CAD build for the part. Positions are in the model's coordinates, mm. Round coordinates to 2 decimals unless told otherwise and drop trailing zeros. Order: outer loops, then holes, each group sorted by start corner. A loop starts at its lowest first (then second) coordinate and runs counter-clockwise, first axis right, second up. Notation, with made-up numbers: M 20.5,57.25 L 39.5,57.25 A23 ccw 39.5,95.25 Z; hole C 37.5,37 d1. An arc over 180 degrees is marked long. Answer as a JSON object with one key per item and string values.
```python
from build123d import *

# Parameters (mm, degrees)
SKETCH1_W                  = 150
SKETCH1_H                  = 260
BOSS_EXTRUDE1_DEPTH        = 10
F_14_0_14_DIAMETER_HOLE1_D = 14


with BuildPart() as part:
    # Sketch1 → Boss-Extrude1 (new body)
    with BuildSketch(Plane.XY):
        Rectangle(SKETCH1_W, SKETCH1_H)
    extrude(amount=BOSS_EXTRUDE1_DEPTH)

    # Ø14.0 (14) Diameter Hole1 (through all)
    with Locations(Plane.XY.offset(10)):
        with Locations((-55, 100), (-55, 0), (-55, -100), (55, -100), (55, 0), (55, 100)):
            Hole(F_14_0_14_DIAMETER_HOLE1_D / 2)


solid = part.part
```
Item 1: Saw through at B-B on z = 7. List the corners of the cut face in (x, y).
Worked answers:
{"outline": "M -75,-130 L 75,-130 L 75,130 L -75,130 Z; hole C -55,-100 d14; hole C -55,0 d14; hole C -55,100 d14; hole C 55,-100 d14; hole C 55,0 d14; hole C 55,100 d14"}
Item 2: Wall check: line 1 along Y through (x, z) = (55, 6); line 2 along Y through (x, z) = (-60.5, 8.5); line 3 along X through (y, z) = (105.5, 6.25). Give the ranges that are in metal, low to high. Write a range as [from, to].
Worked answers:
{"line 1": "y = [-130, -107], [-93, -7], [7, 93], [107, 130]", "line 2": "y = [-130, -104.33], [-95.67, -4.33], [4.33, 95.67], [104.33, 130]", "line 3": "x = [-75, -59.33], [-50.67, 50.67], [59.33, 75]"}
Item 3: Saw through at C-C on x = -55. List the corners of the cut face in (y, z).
Worked answers:
{"outline": "M -130,0 L -107,0 L -107,10 L -130,10 Z; M -93,0 L -7,0 L -7,10 L -93,10 Z; M 7,0 L 93,0 L 93,10 L 7,10 Z; M 107,0 L 130,0 L 130,10 L 107,10 Z"}
Item 4: Saw through at A-A on y = 0. List the corners of the cut face in (x, z).
Worked answers:
{"outline": "M -75,0 L -62,0 L -62,10 L -75,10 Z; M -48,0 L 48,0 L 48,10 L -48,10 Z; M 62,0 L 75,0 L 75,10 L 62,10 Z"}
Item 5: Two-plate mould, pull along Y, no slides. Class faces 1 (the flat face through (-1, 130, 5)), 2 (the cylindrical face through (-54.09, -93.06, 4.93)), 3 (the cylindrical face through (55.91, 106.94, 4.93)), 4 (the flat face through (-75, -2, 5)): released by +Y, released by -Y, zero draft, split by the parting line, or undercut.
Worked answers:
{"face 1": "released by +Y", "face 2": "undercut", "face 3": "undercut", "face 4": "zero draft"}
